CAD build for the part. Positions are in the model's coordinates, mm. A direction names the side the tool comes from. Give positions to 0.01 mm unless a question says otherwise; leave off trailing zeros. Write each loop counter-clockwise with the first axis right and the second up, starting at its lowest first coordinate (ties: lowest second). Pieces come first, ordered by that corner, then holes. Notation, with made-up numbers: (4.25, -2.5) - (14.25, -2.5) arc R21 cw to (14.25, 7.5) - close; hole circle Ø2 at (1, 84.5). An arc over 180 degrees is marked (long way). Put each result on its own line as item: value. Start each with the question number.
1. Cut at D-D on y = -5. List the corners of the cut face in (x, z).
2. Cut at C-C on z = 3.5. List the corners of the cut face in (x, y).
3. Drop flat-ended pins along their axis: pin 1 (2 mm diameter, centred on x = -3.5, z = 5.5, fed in from +Y); pin 2 (3.5 mm diameter, centred on y = -15, z = 6, fed in from +X); pin 3 (6 mm diameter, centred on y = -19.5, z = 5.5, fed in from -X); pin 4 (10 mm diameter, centred on x = -9.5, y = -11.5, fed in from +Z). Give the stop position or say it passes through.
4. Cut at B-B on x = 0. List the corners of the cut face in (y, z), and give its area (3 significant figures).
5. Cut at A-A on y = 0. List the corners of the cut face in (x, z), and give its area (3 significant figures).
6. Mould opens along Y. For faces 1 (the flat face through (0, -23, 12)), 2 (the cylindrical face through (2.17, -9.76, 1.97)), 3 (the flat face through (0, -28, 6)), 4 (the flat face through (0, -24, 6)) say: +Y half, -Y half, draft (parallel to the pull), parting line (faces both ways), or undercut.
7. Tool access for faces 5 (the flat face through (10, -21, 3)), 6 (the flat face through (0, -21, 8)), 7 (the flat face through (0, -18, 10)), 8 (the flat face through (-10, -21, 3)): list every direction of +Z, -Z, +X, -X, +Y, -Y with a clear straight run to the whole face (end or side of a thin tool).
8. Wall check: line 1 (Y direction, x = 0, z = 2.05); line 2 (Z direction, x = 1.5, y = -20); line 3 (X direction, y = -5, z = 3.5). Give the ranges that are in metal, low to high.
from build123d import *

# Parameters (mm, degrees)
BOSS_EXTRUDE1_DEPTH        = 4
SKETCH2_W                  = 20
SKETCH2_H                  = 4
BOSS_EXTRUDE2_DEPTH        = 8
SKETCH3_W                  = 20
SKETCH3_H                  = 4
BOSS_EXTRUDE3_DEPTH        = 6
F_20_0_20_DIAMETER_HOLE1_D = 20


with BuildPart() as part:
    # Sketch1 → Boss-Extrude1 (new body)
    with BuildSketch(Plane(origin=(0, 0, 0), x_dir=(-1, 0, 0), z_dir=(0, 0, -1))):
        with BuildLine():
            Line((-10, -28), (10, -28))
            Line((10, -28), (10, -9.797958971))
            ThreePointArc((10, -9.797958971), (0, 14), (-10, -9.797958971))
            Line((-10, -9.797958971), (-10, -28))
        make_face()
    extrude(amount=-BOSS_EXTRUDE1_DEPTH)

    # Sketch2 → Boss-Extrude2 (add)
    with BuildSketch(Plane.XY.offset(4)):
        with Locations((0, -26)):
            Rectangle(SKETCH2_W, SKETCH2_H)
    extrude(amount=BOSS_EXTRUDE2_DEPTH)

    # Sketch3 → Boss-Extrude3 (add)
    with BuildSketch(Plane(origin=(0, -24, 0), x_dir=(-1, 0, 0), z_dir=(0, 1, 0))):
        with Locations((0, 10)):
            Rectangle(SKETCH3_W, SKETCH3_H)
    extrude(amount=BOSS_EXTRUDE3_DEPTH)

    # Ø20.0 (20) Diameter Hole1 (through all)
    with Locations(Plane.XY.offset(4)):
        with Locations((0, 0)):
            Hole(F_20_0_20_DIAMETER_HOLE1_D / 2)


solid = part.part
Report:
1. outline: (-13.08, 0) - (-8.66, 0) - (-8.66, 4) - (-13.08, 4) - close; (8.66, 0) - (13.08, 0) - (13.08, 4) - (8.66, 4) - close
2. outline: (-10, -28) - (10, -28) - (10, -9.8) arc R14 ccw (long way) to (-10, -9.8) - close; hole circle Ø20 at (0, 0)
3. pin 1: stops at y = -24
3. pin 2: passes through
3. pin 3: stops at x = -10
3. pin 4: stops at z = 4
4. outline: (-28, 0) - (-10, 0) - (-10, 4) - (-24, 4) - (-24, 8) - (-18, 8) - (-18, 12) - (-28, 12) - close; (10, 0) - (14, 0) - (14, 4) - (10, 4) - close
4. area: 144 mm²
5. outline: (-14, 0) - (-10, 0) - (-10, 4) - (-14, 4) - close; (10, 0) - (14, 0) - (14, 4) - (10, 4) - close
5. area: 32.0 mm²
6. face 1: draft
6. face 2: undercut
6. face 3: -Y half
6. face 4: +Y half
7. face 5: +Z, -Z, +X, -Y
7. face 6: +X, -X, +Y
7. face 7: +Z, +X, -X, +Y
7. face 8: +Z, -Z, -X, -Y
8. line 1: y = -28 to -10, 10 to 14
8. line 2: z = 0 to 4, 8 to 12
8. line 3: x = -13.08 to -8.66, 8.66 to 13.08
